from build123d import *

# Parameters (mm, degrees)
SKETCH1_R           = 15
BOSS_EXTRUDE1_DEPTH = 4
SKETCH2_R           = 11.75
BOSS_EXTRUDE2_DEPTH = 6
SKETCH3_R           = 8.5
CUT_EXTRUDE1_DEPTH  = 20
CHAMFER1_SIZE       = 0.5
CHAMFER2_SIZE       = 0.5


with BuildPart() as part:
    # Sketch1 → Boss-Extrude1 (new body)
    with BuildSketch(Plane.XY):
        Circle(SKETCH1_R)
    extrude(amount=BOSS_EXTRUDE1_DEPTH)

    # Sketch2 → Boss-Extrude2 (add)
    with BuildSketch(Plane.XY.offset(4)):
        Circle(SKETCH2_R)
    extrude(amount=BOSS_EXTRUDE2_DEPTH)

    # Sketch3 → Cut-Extrude1 (cut)
    with BuildSketch(Plane(origin=(0, 0, 0), x_dir=(-1, 0, 0), z_dir=(0, 0, -1))):
        Circle(SKETCH3_R)
    extrude(amount=-CUT_EXTRUDE1_DEPTH, mode=Mode.SUBTRACT)

    # Chamfer1
    chamfer1_edges = [part.edges().sort_by_distance(p)[0] for p in [
        (8.5, 0, 10),
        (8.5, 0, 0),
    ]]
    chamfer(chamfer1_edges, length=CHAMFER1_SIZE)

    # Chamfer2
    chamfer2_edges = [part.edges().sort_by_distance(p)[0] for p in [
        (-15, 0, 0),
        (-15, 0, 4),
        (-11.75, 0, 10),
    ]]
    chamfer(chamfer2_edges, length=CHAMFER2_SIZE)


solid = part.part
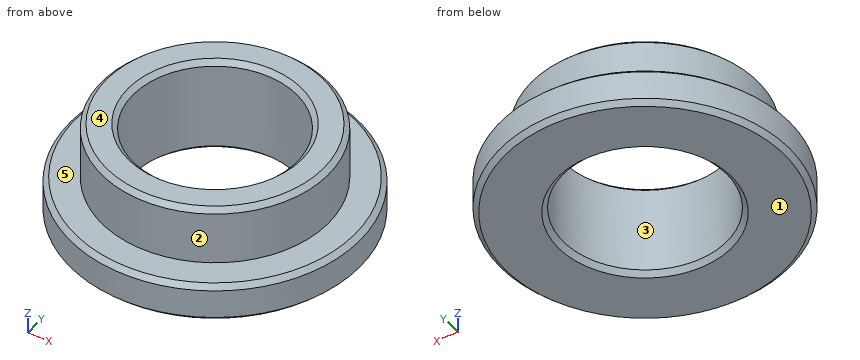
The model under review builds one solid part; all positions refer to its coordinate system, in mm. Face numbers are marked on the shaded views. A direction names the side the tool comes from. Round coordinates to 2 decimals unless told otherwise and drop trailing zeros. Loops run counter-clockwise (first coordinate to the right, second up) from the corner with the lowest first, then second, coordinate; pieces in that order, holes last. Notation, with made-up numbers: (-2.5, 27) -> (26.5, 27) arc R21 cw to (26.5, 58) -> close; hole circle Ø1 at (-28.75, 74.5). An arc over 180 degrees is marked (long way). Answer as CSV lines item,"result".
1) Add section D-D on z = 6.5. Write out the cut boundary in (x, y).
Geometry results:
outline,"circle Ø23.5 at (0, 0); hole circle Ø17 at (0, 0)"
2) To check wall thickness, follow line 1 along Y through (x, z) = (0, 6); line 2 along Y through (x, z) = (0, 2.5); line 3 along X through (y, z) = (4.25, 5). State the ranges of each line that lie inside material, in increasing order. Write a range as from..to.
Geometry results:
line 1,"y = -11.75..-8.5, 8.5..11.75"
line 2,"y = -15..-8.5, 8.5..15"
line 3,"x = -10.95..-7.36, 7.36..10.95"
3) Tool access review of the marked faces 4 and 5: name each direction out of +Z, -Z, +X, -X, +Y, -Y from which nothing blocks a thin tool from reaching the whole face with its end or side.
Geometry results:
face 4,"+Z, +X, -X, +Y, -Y"
face 5,"+Z"
4) For P1, Ø6, axis at y = 6, z = 2, coming from the +X side; P2, Ø6, axis at x = 7.5, z = 1, coming from the +Y side, all flat-tipped, find the tip position at first contact; note any pin that passes through.
Geometry results:
P1,"stops at x = 14.7"
P2,"stops at y = 14.31"
5) Add section C-C on z = 1. Write out the cut boundary in (x, y).
Geometry results:
outline,"circle Ø30 at (0, 0); hole circle Ø17 at (0, 0)"
6) Draft analysis for pull direction X (two halves, no side actions). For the marked faces 1, 2 and 3, state which applies: pulls with the +X half, pulls with the -X half, needs draft (parallel to the pull), parting line crosses it, or undercut.
Geometry results:
face 1,"needs draft"
face 2,"parting line crosses it"
face 3,"undercut"
7) Add section A-A on y = 0. Write out the cut boundary in (x, z).
Geometry results:
outline,"(-15, 0.5) -> (-14.5, 0) -> (-9, 0) -> (-8.5, 0.5) -> (-8.5, 9.5) -> (-9, 10) -> (-11.25, 10) -> (-11.75, 9.5) -> (-11.75, 4) -> (-14.5, 4) -> (-15, 3.5) -> close; (8.5, 0.5) -> (9, 0) -> (14.5, 0) -> (15, 0.5) -> (15, 3.5) -> (14.5, 4) -> (11.75, 4) -> (11.75, 9.5) -> (11.25, 10) -> (9, 10) -> (8.5, 9.5) -> close"
